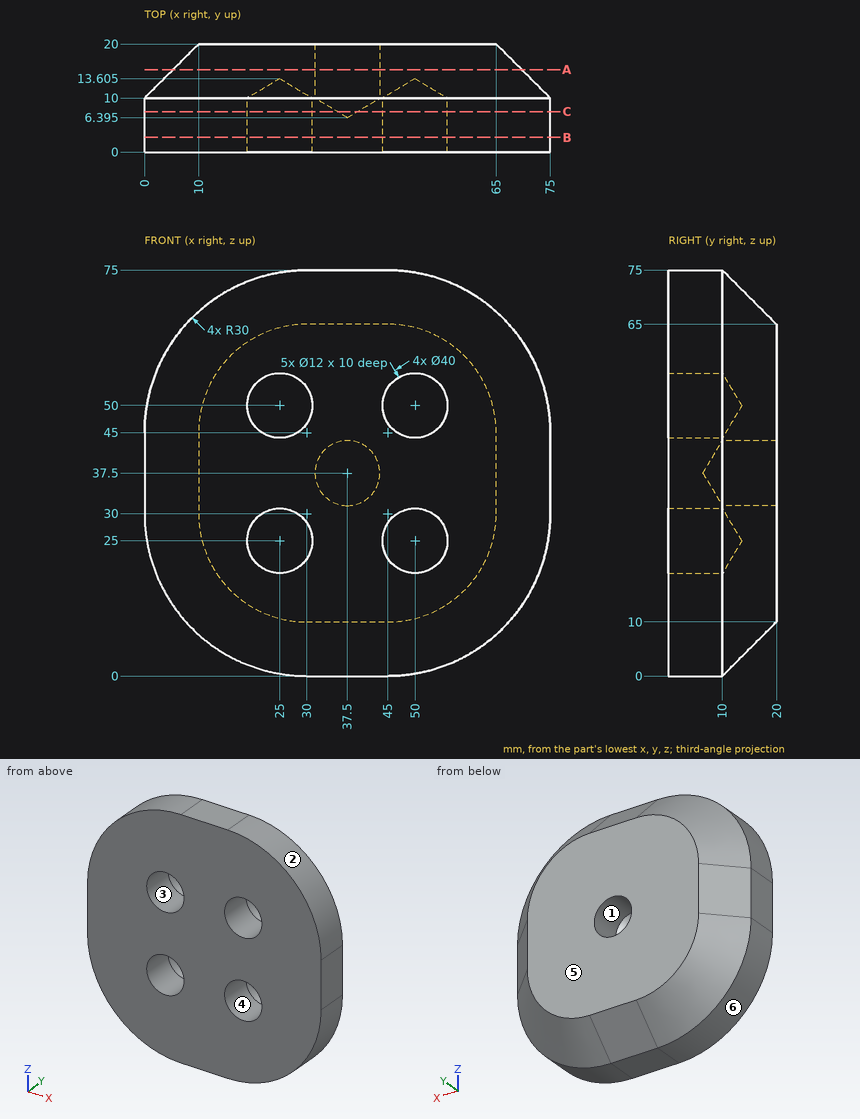
Job drawing, mm, ordinate dimensions from the low corner. One solid piece. A direction names the side the tool comes from. Give positions to 0.01 mm unless a question says otherwise; leave off trailing zeros. Order: outer loops, then holes, each group sorted by start corner. A loop starts at its lowest first (then second) coordinate and runs counter-clockwise, first axis right, second up. Notation, with made-up numbers: M 52.5,75 L 102.5,75 A8 ccw 102.5,79 Z; hole C 44.25,25 d10. An arc over 180 degrees is marked long. Put each result on its own line as item: value. Start each with the question number.
(1) Tool access for the marked faces 1, 2 and 3: list every direction of +Z, -Z, +X, -X, +Y, -Y with a clear straight run to the whole face (end or side of a thin tool).
(2) Drill centre lines: L1, parallel to X at y = 5.75, z = 50; L2, parallel to Z at x = 52, y = 2.75; L3, parallel to Z at x = 24, y = 8.25. Where is each one in solid material? Low to high. Write a range as [from, to].
(3) Band-saw the part on B-B on y = 2.75. Give the cut face in (x, z).
(4) Band-saw the part on A-A on y = 15.25. Give the cut face in (x, z).
(5) Pull direction X, two halves, no side cores. Call the marked faces 4, 5 and 6: released by +X, released by -X, zero draft, split by the parting line, or undercut.
(6) Band-saw the part on C-C on y = 7.5. Give the cut face in (x, z), then the cut area to 3 significant figures.
(7) Pin check, flat tips, straight feed: pin 1 Ø6 at (x, y) = (55, 18) entering from -Z; pin 2 Ø1 at (y, z) = (3, 67) entering from -X; pin 3 Ø11 at (x, z) = (50, 50) entering from -Y. Stop position of each tip, or through.
Results below:
1. face 1: +Y
1. face 2: +Z, +X, +Y, -Y
1. face 3: -Y
2. L1: x = [0.42, 19], [31, 44], [56, 74.58]
2. L2: z = [0.83, 19.34], [30.66, 44.34], [55.66, 74.17]
2. L3: z = [0.61, 19.08], [30.92, 44.08], [55.92, 74.39]
3. outline: M 0,30 A30 ccw 30,0 L 45,0 A30 ccw 75,30 L 75,45 A30 ccw 45,75 L 30,75 A30 ccw 0,45 Z; hole C 25,25 d12; hole C 25,50 d12; hole C 50,25 d12; hole C 50,50 d12
4. outline: M 5.25,30 A24.75 ccw 30,5.25 L 45,5.25 A24.75 ccw 69.75,30 L 69.75,45 A24.75 ccw 45,69.75 L 30,69.75 A24.75 ccw 5.25,45 Z; hole C 37.5,37.5 d12
5. face 4: undercut
5. face 5: zero draft
5. face 6: released by -X
6. outline: M 0,30 A30 ccw 30,0 L 45,0 A30 ccw 75,30 L 75,45 A30 ccw 45,75 L 30,75 A30 ccw 0,45 Z; hole C 25,25 d12; hole C 25,50 d12; hole C 37.5,37.5 d3.68; hole C 50,25 d12; hole C 50,50 d12
6. area: 4,390 mm2
7. pin 1: stops at z = 6.86
7. pin 2: stops at x = 9.08
7. pin 3: stops at y = 10.3
